```python
from build123d import *


with BuildPart() as part:
    # Sketch1 → Revolve1 (revolve)
    with BuildSketch(Plane.XY):
        Polygon((0, 4.5), (0, 0.5), (5.5, 0.5), (8, 3), (8, 7.5), (4, 7.5), (4, 4.5), align=None)
    revolve(axis=Axis((8, 0, 0), (-1, 0, 0)))


solid = part.part
```
Model file for the job. Use its own axes, mm. A direction names the side the tool comes from. Give positions to 0.01 mm unless a question says otherwise; leave off trailing zeros. Loops run counter-clockwise (first coordinate to the right, second up) from the corner with the lowest first, then second, coordinate; pieces in that order, holes last. Notation, with made-up numbers: M 8,13.25 L 41,13.25 A19 ccw 41,40.25 Z; hole C 5.5,6 d5. An arc over 180 degrees is marked long. Use one line per item in the form item = value.
Item 1: Slice it at A-A on z = 0. List the corners of the cut face in (x, y), and give its area (4 significant figures).
Filled in:
outline = M 0,-4.5 L 4,-4.5 L 4,-7.5 L 8,-7.5 L 8,-3 L 5.5,-0.5 L 0,-0.5 Z; M 0,0.5 L 5.5,0.5 L 8,3 L 8,7.5 L 4,7.5 L 4,4.5 L 0,4.5 Z
area = 81.75 mm^2
Item 2: Flat gauge pins, fed straight in: pin 1 Ø1.5 at (x, z) = (3, 2.5) entering from -Y; pin 2 Ø4 at (x, y) = (3, -2) entering from +Z; pin 3 Ø1.5 at (x, z) = (6.5, 3.5) entering from +Y. Where does each tip first touch, or does it go through?
Filled in:
pin_1 = -4.15
pin_2 = 7.5
pin_3 = 6.98
Item 3: Drill centre lines: L1, parallel to Z at x = 2.6, y = 0; L2, parallel to Y at x = 4.25, z = 0. Where is each one in solid material? Low to high.
Filled in:
L1 = -4.5 to -0.5, 0.5 to 4.5
L2 = -7.5 to -0.5, 0.5 to 7.5
Item 4: Slice it at C-C on x = 1. List the corners of the cut face in (y, z).
Filled in:
outline = C 0,0 d9; hole C 0,0 d1
Item 5: Slice it at D-D on y = 3.75. List the corners of the cut face in (x, z).
Filled in:
outline = M 0,-2.49 L 4,-2.49 L 4,-6.5 L 8,-6.5 L 8,6.5 L 4,6.5 L 4,2.49 L 0,2.49 Z
Item 6: Two-plate mould, pull along Y, no slides. Class faces 1 (the flat face through (8, 0.1, 3.2)), 2 (the conical face through (6, 1, 0)), 3 (the cylindrical face through (5.972, -7.493, -0.33)): released by +Y, released by -Y, zero draft, split by the parting line, or undercut.
Filled in:
face_1 = zero draft
face_2 = undercut
face_3 = split by the parting line
Item 7: Which spindle directions (+Z, -Z, +X, -X, +Y, -Y) get a long thin tool onto all of the face, cutting with end or side? Do faces 4 (the cylindrical face through (1.97, -0.59, -4.46)), 5 (the cylindrical face through (2.788, -0.108, 0.488)). Say none if no direction does.
Filled in:
face_4 = -X
face_5 = +X, -X
